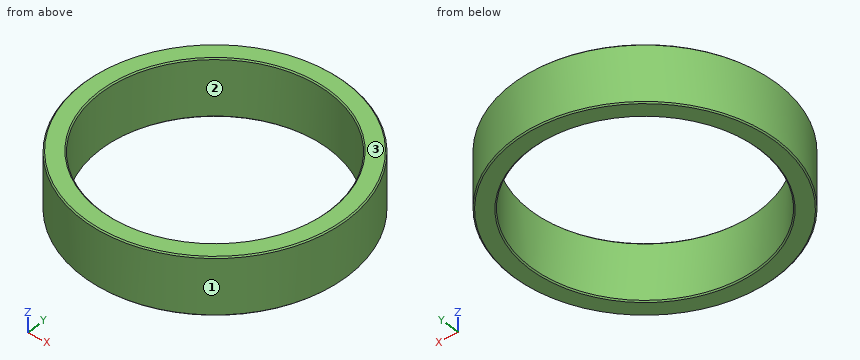
from build123d import *

# Parameters (mm, degrees)
SKETCH1_R           = 55
SKETCH1_R_2         = 47.5
BOSS_EXTRUDE1_DEPTH = 24
CHAMFER1_SIZE       = 0.5


with BuildPart() as part:
    # Sketch1 → Boss-Extrude1 (new body)
    with BuildSketch(Plane.XY):
        Circle(SKETCH1_R)
        Circle(SKETCH1_R_2, mode=Mode.SUBTRACT)
    extrude(amount=BOSS_EXTRUDE1_DEPTH)

    # Chamfer1
    chamfer1_edges = [part.edges().sort_by_distance(p)[0] for p in [
        (-55, 0, 0),
        (-55, 0, 24),
        (-47.5, 0, 0),
        (-47.5, 0, 24),
    ]]
    chamfer(chamfer1_edges, length=CHAMFER1_SIZE)


solid = part.part
CAD build for the part. Positions are in the model's coordinates, mm. Face numbers are marked on the shaded views. Round coordinates to 2 decimals unless told otherwise and drop trailing zeros. Order: outer loops, then holes, each group sorted by start corner. A loop starts at its lowest first (then second) coordinate and runs counter-clockwise, first axis right, second up. Notation, with made-up numbers: (14.25, 76) -> (29.25, 76) arc R26 cw to (29.25, 95) -> close; hole circle Ø11 at (-22.75, -33.5). An arc over 180 degrees is marked (long way). Write item = value, one per line. Start each with the question number.
(1) Pin check, flat tips, straight feed: P1, Ø1, axis at y = 4.5, z = 6.5, coming from the -X side; P2, Ø8, axis at x = -10.5, y = 41.5, coming from the +Z side; P3, Ø12, axis at y = 8.5, z = 14.5, coming from the +X side; P4, Ø6, axis at x = 12.5, z = 18, coming from the -Y side. Stop position of each tip, or through.
(2) Cut at C-C, the plane z = 20.5. List the corners of the cut face in (x, y).
(3) Pull direction X, two halves, no side cores. Call the marked faces 1, 2 and 3: released by +X, released by -X, zero draft, split by the parting line, or undercut.
(4) Cut at A-A, the plane y = 0. List the corners of the cut face in (x, z).
(5) Probe line 1 (Y direction, x = 0, z = 18); line 2 (Y direction, x = -12.5, z = 3.5); line 3 (X direction, y = 26, z = 22). List the from-to ranges inside material, lowest first. Write a range as [from, to].
Model answer:
q1.P1 = -54.85
q1.P2 = through
q1.P3 = 54.94
q1.P4 = -54.17
q2.outline = circle Ø110 at (0, 0); hole circle Ø95 at (0, 0)
q3.face_1 = split by the parting line
q3.face_2 = undercut
q3.face_3 = zero draft
q4.outline = (-55, 0.5) -> (-54.5, 0) -> (-48, 0) -> (-47.5, 0.5) -> (-47.5, 23.5) -> (-48, 24) -> (-54.5, 24) -> (-55, 23.5) -> close; (47.5, 0.5) -> (48, 0) -> (54.5, 0) -> (55, 0.5) -> (55, 23.5) -> (54.5, 24) -> (48, 24) -> (47.5, 23.5) -> close
q5.line_1 = [-55, -47.5], [47.5, 55]
q5.line_2 = [-53.56, -45.83], [45.83, 53.56]
q5.line_3 = [-48.47, -39.75], [39.75, 48.47]
